Geometry check sheet. Reference: the model listing, model coordinates, mm. A direction names the side the tool comes from. Give positions to 0.01 mm unless a question says otherwise; leave off trailing zeros. Loops run counter-clockwise (first coordinate to the right, second up) from the corner with the lowest first, then second, coordinate; pieces in that order, holes last. Notation, with made-up numbers: (82.25, -10) -> (135.25, -10) arc R13 ccw to (135.25, -2) -> close; hole circle Ø8 at (72, 28). An arc over 180 degrees is marked (long way). Answer as a JSON object with one key per item and string values.
from build123d import *

# Parameters (mm, degrees)
SKETCH1_W           = 15
SKETCH1_H           = 22
SKETCH1_R           = 3
BOSS_EXTRUDE1_DEPTH = 8
SKETCH2_W           = 10
SKETCH2_H           = 19
CUT_EXTRUDE1_DEPTH  = 24.34523506
FILLET1_R           = 2
SKETCH3_R           = 3
CUT_EXTRUDE2_DEPTH  = 18


with BuildPart() as part:
    # Sketch1 → Boss-Extrude1 (new, symmetric)
    with BuildSketch(Plane.XY):
        with Locations((0, 5)):
            Rectangle(SKETCH1_W, SKETCH1_H)
        Circle(SKETCH1_R, mode=Mode.SUBTRACT)
    extrude(amount=BOSS_EXTRUDE1_DEPTH, both=True)

    # Sketch2 → Cut-Extrude1 (cut, through all)
    with BuildSketch(Plane(origin=(7.5, 0, 0), x_dir=(0, 0, -1), z_dir=(1, 0, 0))):
        with Locations((0, 3.5)):
            Rectangle(SKETCH2_W, SKETCH2_H)
    extrude(amount=-CUT_EXTRUDE1_DEPTH, mode=Mode.SUBTRACT)

    # Fillet1
    fillet1_edges = [part.edges().sort_by_distance(p)[0] for p in [
        (0, 16, 8),
        (0, 13, 5),
        (0, 13, -5),
        (0, 16, -8),
    ]]
    fillet(fillet1_edges, radius=FILLET1_R)

    # Sketch3 → Cut-Extrude2 (cut)
    with BuildSketch(Plane(origin=(0, 16, 0), x_dir=(1, 0, 0), z_dir=(0, 1, 0))):
        with Locations(Location((0, 0, 0), (0, 0, 270))):
            Circle(SKETCH3_R)
    extrude(amount=-CUT_EXTRUDE2_DEPTH, mode=Mode.SUBTRACT)


solid = part.part
1) Section check C-C on y = -3.5. Record the cut outline in (x, z), plus the area to 3 significant figures.
Geometry check:
{"outline": "(-7.5, -8) -> (7.5, -8) -> (7.5, -5) -> (-7.5, -5) -> close; (-7.5, 5) -> (7.5, 5) -> (7.5, 8) -> (-7.5, 8) -> close", "area": "90.0 mm2"}
2) Depth check by flat-ended pin: P1, Ø1.5, axis at x = 1, z = -3.5, coming from the -Y side; P2, Ø6.5, axis at x = 4, z = 1.5, coming from the -Y side; P3, Ø3, axis at x = -3, z = 1, coming from the -Y side. Enter the tip coordinate at first touch or a pass-through.
Geometry check:
{"P1": "stops at y = 12.56", "P2": "stops at y = 11.97", "P3": "stops at y = 13"}
3) Section check B-B on y = 0. Record the cut outline in (x, z).
Geometry check:
{"outline": "(-7.5, -8) -> (-3, -8) -> (-3, -5) -> (-7.5, -5) -> close; (-7.5, 5) -> (-3, 5) -> (-3, 8) -> (-7.5, 8) -> close; (3, -8) -> (7.5, -8) -> (7.5, -5) -> (3, -5) -> close; (3, 5) -> (7.5, 5) -> (7.5, 8) -> (3, 8) -> close"}
4) Section check A-A on z = 0. Record the cut outline in (x, y), plus the area to 3 significant figures.
Geometry check:
{"outline": "(-7.5, 13) -> (-3, 13) -> (-3, 16) -> (-7.5, 16) -> close; (3, 13) -> (7.5, 13) -> (7.5, 16) -> (3, 16) -> close", "area": "27.0 mm2"}
5) Draft check along Z on faces 3 (the face through (0, -6, -6)), 4 (the face through (5, 13, 0)), 5 (the face through (0.11, 15.4, 7.43)). Enter one of: pulls with the +Z half, pulls with the -Z half, needs draft (parallel to the pull), parting line crosses it, or undercut.
Geometry check:
{"face 3": "needs draft", "face 4": "undercut", "face 5": "pulls with the +Z half"}
6) Material ranges on line 1 along Z through (x, y) = (0, 14); line 2 along Y through (x, z) = (0, -6.05); line 3 along Z through (x, y) = (2, 11), recorded low to high. Write a range as from..to.
Geometry check:
{"line 1": "z = -8..-3, 3..8", "line 2": "y = -6..-3, 3..16", "line 3": "z = -8..-5, 5..8"}
7) Section check D-D on x = 0.75. Record the cut outline in (y, z), plus the area to 3 significant figures.
Geometry check:
{"outline": "(-6, -8) -> (-2.9, -8) -> (-2.9, -5) -> (-6, -5) -> close; (-6, 5) -> (-2.9, 5) -> (-2.9, 8) -> (-6, 8) -> close; (2.9, -8) -> (14, -8) arc R2 ccw to (16, -6) -> (16, -2.9) -> (13, -2.9) -> (13, -3) arc R2 cw to (11, -5) -> (2.9, -5) -> close; (2.9, 5) -> (11, 5) arc R2 cw to (13, 3) -> (13, 2.9) -> (16, 2.9) -> (16, 6) arc R2 ccw to (14, 8) -> (2.9, 8) -> close", "area": "110 mm2"}
8) Tool access check on faces 1 (the face through (0, 4, 5)), 2 (the face through (7.5, 4.8, 5.4)). Record the directions out of +Z, -Z, +X, -X, +Y, -Y that give a thin tool (end or side, any length) a straight path to the whole face; none if there is none.
Geometry check:
{"face 1": "+X, -X, -Y", "face 2": "+Z, -Z, +X, +Y, -Y"}
